Here's the drawing with two shaded views (mm, measured from the low corner). I have some questions. Coordinates: 2 decimals unless noted, no trailing zeros. Loops run counter-clockwise (first coordinate to the right, second up) from the corner with the lowest first, then second, coordinate; pieces in that order, holes last. Notation, with made-up numbers: (79, -6) - (89, -6) arc R7 ccw to (89, 1) - close; hole circle Ø4 at (71, 23). An arc over 180 degrees is marked (long way). One line per item, written item: value. Start each with the question number.
(1) If we section it at A-A on y = 25.4: Write out the boundary of the cut face in (x, z) (1 decimal), then the cut area to 3 significant figures.
(2) If I drill on line 1 along X through (y, z) = (24.5, 5.75); line 2 along X through (y, z) = (20, 5.25); line 3 along Y through (x, z) = (133, 1), over which ranges is the centre line in solid material (lowest first)? Write a range as from..to.
(3) I'm going to push flat-ended pins straight in: P1, Ø5, axis at x = 75.5, y = 45, coming from the -Z side; P2, Ø11.5, axis at x = 15.875, y = 25.4, coming from the +Z side. Where does each tip first touch, or does it pass through?
(4) If we section it at D-D on y = 14.5: Write out the boundary of the cut face in (x, z), then the cut area to 3 significant figures.
(5) If we section it at C-C on x = 129: Write out the boundary of the cut face in (y, z).
(6) If we section it at B-B on z = 2.5: Count the separate pieces of the cut face and the enclosed holes in it, then the cut area to 3 significant figures.
(7) If we mould it in two halves opening along X, with no side actions, what happens to the marked faces 1, 2 and 3? For each: pulls with the +X half, pulls with the -X half, needs draft (parallel to the pull), parting line crosses it, or undercut.
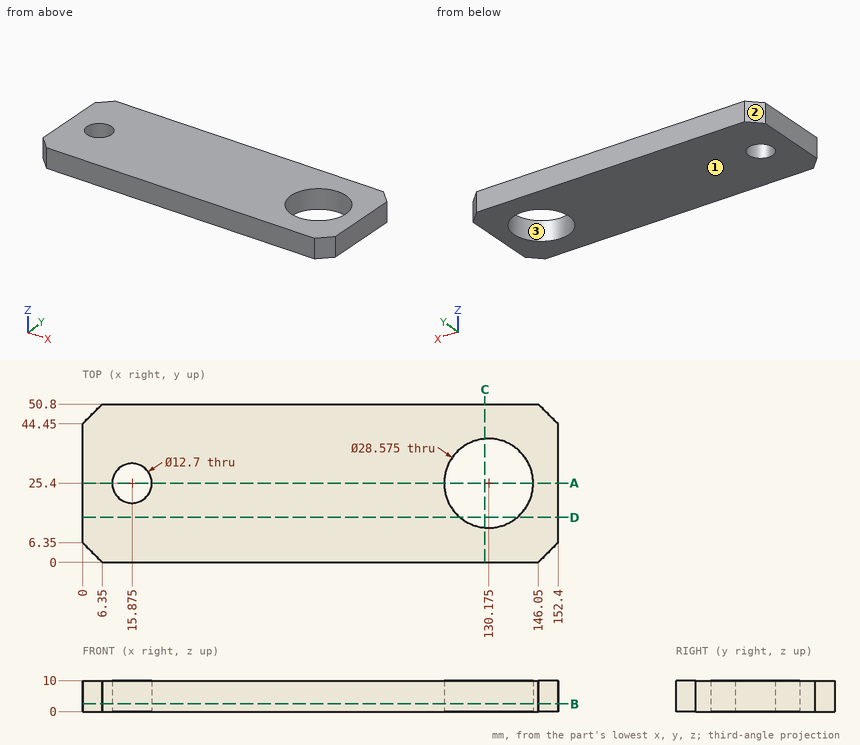
Values:
1. outline: (0, 0) - (9.5, 0) - (9.5, 10) - (0, 10) - close; (22.2, 0) - (115.9, 0) - (115.9, 10) - (22.2, 10) - close; (144.5, 0) - (152.4, 0) - (152.4, 10) - (144.5, 10) - close
1. area: 1,110 mm2
2. line 1: x = 0..9.59, 22.16..115.92, 144.43..152.4
2. line 2: x = 0..12.53, 19.22..116.95, 143.4..152.4
2. line 3: y = 0..11.39, 39.41..50.8
3. P1: stops at z = 0
3. P2: passes through
4. outline: (0, 0) - (120.94, 0) - (120.94, 10) - (0, 10) - close; (139.41, 0) - (152.4, 0) - (152.4, 10) - (139.41, 10) - close
4. area: 1,340 mm2
5. outline: (0, 0) - (11.16, 0) - (11.16, 10) - (0, 10) - close; (39.64, 0) - (50.8, 0) - (50.8, 10) - (39.64, 10) - close
6. separate pieces: 1
6. enclosed holes: 2
6. area: 6,890 mm2
7. face 1: needs draft
7. face 2: pulls with the -X half
7. face 3: undercut
